Work out the finished part from the listing and answer in its coordinate system (mm). A direction names the side the tool comes from. Give positions to 0.01 mm unless a question says otherwise; leave off trailing zeros. Loops run counter-clockwise (first coordinate to the right, second up) from the corner with the lowest first, then second, coordinate; pieces in that order, holes last. Notation, with made-up numbers: (83.5, 50.5) -> (140.5, 50.5) arc R20 ccw to (140.5, 59.5) -> close; hole circle Ø1 at (-29, 5.25). An arc over 180 degrees is marked (long way). Answer as CSV lines item,"result". Start each with the question number.
1. Find the intervals of material crossed by line 1 along Y through (x, z) = (-25, -2.6); line 2 along Y through (x, z) = (67, 3.2); line 3 along X through (y, z) = (-80, -2.5), in increasing order.
2. Find section A-A, the plane y = 25. Give the vertices of the cut face in (x, z), and give its area (4 significant figures).
3. Find section B-B, the plane x = 67. Give the vertices of the cut face in (y, z), and give its area (4 significant figures).
4. A tool of negligible diameter and unlimited length cuts with its end or side. For faces 1 (the face through (24.133, 63.095, 2.535)), 2 (the face through (-1, 100, 0)), from which of +Z, -Z, +X, -X, +Y, -Y can it reach the whole face along a straight path? Write none if from no direction.
5. Find section C-C, the plane z = 2. Count the separate pieces of the cut face and the enclosed holes in it, and give its area (3 significant figures).
6. Determine the mould class of faces 3 (the face through (-74, -98, 0)), 4 (the face through (73, 99, 0)), 5 (the face through (25.488, -69.196, -2.535)) for opening direction Y: +Y half, -Y half, draft (parallel to the pull), parting line (faces both ways), or undercut.
7. A flat-ended cylindrical pin translates along its axis: pin 1 Ø6 at (x, y) = (-25, 67) entering from +Z. Find the tip coordinate at first contact, or state that the pin passes through.
from build123d import *

# Parameters (mm, degrees)
SKETCH_1_W                  = 150
SKETCH_1_H                  = 200
SKETCH_1_R                  = 2
EXTRUDE_1_DEPTH             = 5
SKETCH_2_R                  = 4
CUT_EXTRUDE_1_DEPTH         = 4.5
HOLE_WIZARD_M4_1_D          = 3.3
HOLE_WIZARD_1_D             = 4.5
HOLE_WIZARD_1_CBORE_D       = 8
HOLE_WIZARD_1_CBORE_DEPTH   = 5
SKETCH_7_R                  = 4.920568007
SKETCH_7_R_2                = 5.393736445
SKETCH_7_R_3                = 5.34126294
SKETCH_7_R_4                = 5.362446972
EXTRUDE_2_DEPTH             = 10
FILLET_1_R                  = 5
HOLE_WIZARD_2_D             = 4.5
HOLE_WIZARD_2_CBORE_D       = 8
HOLE_WIZARD_2_CBORE_DEPTH   = 5
PATTERN_LINEAR_2_COUNT      = 4
PATTERN_LINEAR_2_PITCH      = 40
PATTERN_LINEAR_2_COUNT_DIR2 = 5
PATTERN_LINEAR_2_PITCH_DIR2 = 40


with BuildPart() as part:
    # 草图1 → 凸台-拉伸1 (new, symmetric)
    with BuildSketch(Plane.XY):
        Rectangle(SKETCH_1_W, SKETCH_1_H)
        with Locations((-67, 25)):
            Circle(SKETCH_1_R, mode=Mode.SUBTRACT)
        with Locations(Location((-67, -25, 0), (0, 0, 180))):
            Circle(SKETCH_1_R, mode=Mode.SUBTRACT)
        with Locations((67, -25)):
            Circle(SKETCH_1_R, mode=Mode.SUBTRACT)
        with Locations(Location((67, 25, 0), (0, 0, 180))):
            Circle(SKETCH_1_R, mode=Mode.SUBTRACT)
    extrude(amount=EXTRUDE_1_DEPTH, both=True)

    # 草图2 → 切除-拉伸1 (cut)
    with BuildSketch(Plane.XY.offset(5)):
        with Locations((67, 25)):
            Circle(SKETCH_2_R)
        with Locations((67, -25)):
            Circle(SKETCH_2_R)
        with Locations((-67, -25)):
            Circle(SKETCH_2_R)
        with Locations((-67, 25)):
            Circle(SKETCH_2_R)
    extrude(amount=-CUT_EXTRUDE_1_DEPTH, mode=Mode.SUBTRACT)

    # M4 螺纹孔1 (through all)
    with Locations(Plane.XY.offset(5)):
        with Locations((-60, 80)):
            hole_wizard_m4_1 = Hole(HOLE_WIZARD_M4_1_D / 2)

    # 打孔尺寸(%根据)开槽圆柱头螺钉的类型1 (through all)
    with Locations(Plane.XY.offset(5)):
        with Locations((-25, 67), (25, 67), (-25, -67), (25, -67)):
            CounterBoreHole(HOLE_WIZARD_1_D / 2, HOLE_WIZARD_1_CBORE_D / 2, HOLE_WIZARD_1_CBORE_DEPTH)

    # 草图7 → 凸台-拉伸2 (add)
    with BuildSketch(Plane.XY.offset(5)):
        with Locations((-67, 25)):
            Circle(SKETCH_7_R)
        with Locations((-67, -25)):
            Circle(SKETCH_7_R_2)
        with Locations((67, -25)):
            Circle(SKETCH_7_R_3)
        with Locations((67, 25)):
            Circle(SKETCH_7_R_4)
    extrude(amount=-EXTRUDE_2_DEPTH)

    # 圆角1
    fillet_1_edges = [part.edges().sort_by_distance(p)[0] for p in [
        (75, -100, 0),
        (-75, -100, 0),
        (-75, 100, 0),
        (75, 100, 0),
    ]]
    fillet(fillet_1_edges, radius=FILLET_1_R)

    # 打孔尺寸(%根据)开槽圆柱头螺钉的类型2 (through all)
    with Locations(Plane.XY.offset(5)):
        with Locations((-67, 25), (67, 25), (-67, -25), (67, -25)):
            CounterBoreHole(HOLE_WIZARD_2_D / 2, HOLE_WIZARD_2_CBORE_D / 2, HOLE_WIZARD_2_CBORE_DEPTH)

    # 阵列(线性)2: Hole Wizard M4 _1 4 × 5
    with Locations(*[(i * PATTERN_LINEAR_2_PITCH, -j * PATTERN_LINEAR_2_PITCH_DIR2, 0) for i in range(PATTERN_LINEAR_2_COUNT) for j in range(PATTERN_LINEAR_2_COUNT_DIR2) if (i, j) != (0, 0)]):
        add(hole_wizard_m4_1, mode=Mode.SUBTRACT)


solid = part.part
Resolved:
1,line 1,"y = -100 to -69.25, -64.75 to 64.75, 69.25 to 100"
1,line 2,"y = -100 to -29, -21 to 21, 29 to 100"
1,line 3,"x = -75 to -61.65, -58.35 to -21.65, -18.35 to 18.35, 21.65 to 58.35, 61.65 to 75"
2,outline,"(-75, -5) -> (-69.25, -5) -> (-69.25, 0) -> (-71, 0) -> (-71, 5) -> (-75, 5) -> close; (-64.75, -5) -> (64.75, -5) -> (64.75, 0) -> (63, 0) -> (63, 5) -> (-63, 5) -> (-63, 0) -> (-64.75, 0) -> close; (69.25, -5) -> (75, -5) -> (75, 5) -> (71, 5) -> (71, 0) -> (69.25, 0) -> close"
2,area,"1,375 mm^2"
3,outline,"(-100, -5) -> (-27.25, -5) -> (-27.25, 0) -> (-29, 0) -> (-29, 5) -> (-100, 5) -> close; (-22.75, -5) -> (22.75, -5) -> (22.75, 0) -> (21, 0) -> (21, 5) -> (-21, 5) -> (-21, 0) -> (-22.75, 0) -> close; (27.25, -5) -> (100, -5) -> (100, 5) -> (29, 5) -> (29, 0) -> (27.25, 0) -> close"
3,area,"1,875 mm^2"
4,face 1,"+Z"
4,face 2,"+Z, -Z, +X, -X, +Y"
5,separate pieces,"1"
5,enclosed holes,"28"
5,area,"29,400 mm^2"
6,face 3,"-Y half"
6,face 4,"+Y half"
6,face 5,"undercut"
7,pin 1,"stops at z = 0"
